```python
from build123d import *

# Parameters (mm, degrees)
SKETCH1_R           = 30
BOSS_EXTRUDE1_DEPTH = 40


with BuildPart() as part:
    # Sketch1 → Boss-Extrude1 (new body)
    with BuildSketch(Plane.XY):
        with BuildLine():
            Line((0, 0), (300, 0))
            Line((300, 0), (212.744219232, 533.229771362))
            ThreePointArc((212.744219232, 533.229771362), (205.956719326, 545.241316007), (193.006727574, 550))
            Line((193.006727574, 550), (106.993272426, 550))
            ThreePointArc((106.993272426, 550), (94.043280674, 545.241316007), (87.255780768, 533.229771362))
            Line((87.255780768, 533.229771362), (0, 0))
        make_face()
        with Locations((150, 486)):
            Circle(SKETCH1_R, mode=Mode.SUBTRACT)
    extrude(amount=BOSS_EXTRUDE1_DEPTH)


solid = part.part
```
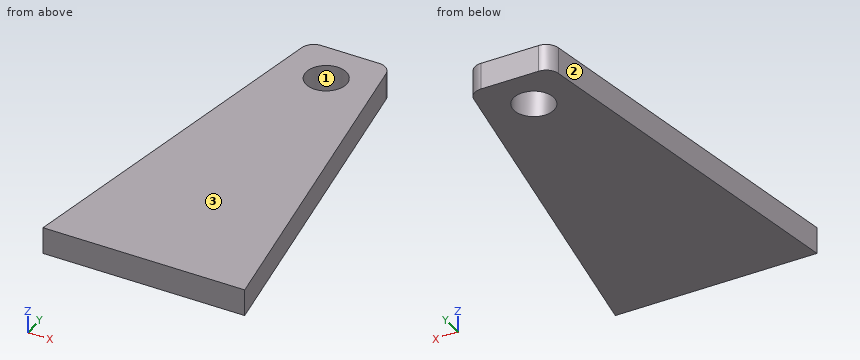
Could you check a few things on this model? Use its own coordinates, in mm. Face numbers are marked on the shaded views. Give positions to 0.01 mm unless a question says otherwise; leave off trailing zeros. Loops run counter-clockwise (first coordinate to the right, second up) from the corner with the lowest first, then second, coordinate; pieces in that order, holes last. Notation, with made-up numbers: (49.25, 33) -> (82.25, 33) arc R26 cw to (82.25, 62) -> close; hole circle Ø1 at (79, -23.5). An arc over 180 degrees is marked (long way). Put each result on its own line as item: value.
(1) Imagine slicing it at A-A on x = 150. Write out the boundary of the cut face in (y, z).
Computed:
outline: (0, 0) -> (456, 0) -> (456, 40) -> (0, 40) -> close; (516, 0) -> (550, 0) -> (550, 40) -> (516, 40) -> close
(2) Imagine slicing it at B-B on y = 476. Write out the boundary of the cut face in (x, z), plus the area to 3 significant figures.
Computed:
outline: (77.89, 0) -> (121.72, 0) -> (121.72, 40) -> (77.89, 40) -> close; (178.28, 0) -> (222.11, 0) -> (222.11, 40) -> (178.28, 40) -> close
area: 3,510 mm^2
(3) I'm going to push flat-ended pins straight in: pin 1 Ø1.5 at (y, z) = (200.5, 7) entering from -X; pin 2 Ø6 at (y, z) = (149.5, 35) entering from -X; pin 3 Ø1.5 at (y, z) = (405.5, 18.5) entering from -X. Where does each tip first touch, or does it pass through?
Computed:
pin 1: x = 32.69
pin 2: x = 23.97
pin 3: x = 66.23
(4) Thinking about a two-plate mould opening in Y: for the marked faces 1, 2 and 3, which applies, pulls with the +Y half, pulls with the -Y half, needs draft (parallel to the pull), parting line crosses it, or undercut?
Computed:
face 1: undercut
face 2: pulls with the +Y half
face 3: needs draft
(5) Imagine slicing it at C-C on z = 34.5. Write out the boundary of the cut face in (x, y).
Computed:
outline: (0, 0) -> (300, 0) -> (212.74, 533.23) arc R20 ccw to (193.01, 550) -> (106.99, 550) arc R20 ccw to (87.26, 533.23) -> close; hole circle Ø60 at (150, 486)
(6) Imagine slicing it at D-D on x = 250.5. Write out the boundary of the cut face in (y, z), plus the area to 3 significant figures.
Computed:
outline: (0, 0) -> (302.5, 0) -> (302.5, 40) -> (0, 40) -> close
area: 12,100 mm^2
(7) Please list where these lines run through material, in increasing order: probe 1 along Y at (x, z) = (150, 20.5); probe 2 along Y at (x, z) = (128, 22); probe 3 along X at (y, z) = (488, 37). Write a range as [from, to].
Computed:
probe 1: [0, 456], [516, 550]
probe 2: [0, 465.6], [506.4, 550]
probe 3: [79.85, 120.07], [179.93, 220.15]
